The listing builds one solid part. Answer for the finished solid, in the listing's coordinates (mm). A direction names the side the tool comes from. Coordinates: 2 decimals unless noted, no trailing zeros. Order: outer loops, then holes, each group sorted by start corner. A loop starts at its lowest first (then second) coordinate and runs counter-clockwise, first axis right, second up.
```python
from build123d import *

# Parameters (mm, degrees)
BASE_FLANGE_SKETCH_R = 8
BASE_FLANGE_DEPTH    = 9
TOWER_DEPTH          = 30
SIDE_SLOT_DEPTH      = 21
CLIP_BOSS_DEPTH      = 6
CLIP_BOSS_DEPTH_BACK = 1
CLIP_SLOT_REACH      = 174.171
CLIP_SLOT_END_RADIUS = 15


with BuildPart() as part:
    # Base Flange Sketch → Base Flange (new body)
    with BuildSketch(Plane(origin=(0, 0, 0), x_dir=(1, 0, 0), z_dir=(0, 1, 0))):
        with BuildLine():
            Line((-27, 40), (27, 40))
            ThreePointArc((27, 40), (49.192388155, 49.192388155), (40, 27))
            Line((40, 27), (40, -27))
            ThreePointArc((40, -27), (49.192388155, -49.192388155), (27, -40))
            Line((27, -40), (-27, -40))
            ThreePointArc((-27, -40), (-49.192388155, -49.192388155), (-40, -27))
            Line((-40, -27), (-40, 27))
            ThreePointArc((-40, 27), (-49.192388155, 49.192388155), (-27, 40))
        make_face()
        with Locations(Location((-40, 40, 0), (0, 0, 270))):
            Circle(BASE_FLANGE_SKETCH_R, mode=Mode.SUBTRACT)
        with Locations(Location((40, 40, 0), (0, 0, 270))):
            Circle(BASE_FLANGE_SKETCH_R, mode=Mode.SUBTRACT)
        with Locations(Location((40, -40, 0), (0, 0, 270))):
            Circle(BASE_FLANGE_SKETCH_R, mode=Mode.SUBTRACT)
        with Locations(Location((-40, -40, 0), (0, 0, 270))):
            Circle(BASE_FLANGE_SKETCH_R, mode=Mode.SUBTRACT)
    extrude(amount=BASE_FLANGE_DEPTH)

    # Tower Profile Sketch → Tower (add, symmetric)
    with BuildSketch(Plane(origin=(0, 0, 0), x_dir=(0, 0, -1), z_dir=(1, 0, 0))):
        with BuildLine():
            Line((-30, 9), (-30, 125))
            ThreePointArc((-30, 125), (-21.213203436, 146.213203436), (0, 155))
            Line((0, 155), (0, 45))
            Line((0, 45), (30, 45))
            Line((30, 45), (30, 9))
            Line((30, 9), (-30, 9))
        make_face()
    extrude(amount=TOWER_DEPTH, both=True)

    # Lower Bore Profile Sketch → Lower Bore (revolve, cut)
    with BuildSketch(Plane(origin=(0, 0, 0), x_dir=(-1, 0, 0), z_dir=(0, 0, -1))):
        Polygon((30, 134), (10, 134), (10, 140), (-10, 140), (-10, 145), (-30, 145), (-30, 125), (30, 125), align=None)
    revolve(axis=Axis((30, 125, 0), (-1, 0, 0)), mode=Mode.SUBTRACT)

    # Upper Bore Profile Sketch → Upper Bore (revolve, cut)
    with BuildSketch(Plane(origin=(0, 0, 0), x_dir=(-1, 0, 0), z_dir=(0, 0, -1))):
        Polygon((30, 57), (15, 57), (15, 52), (-10, 52), (-10, 57), (-30, 57), (-30, 45), (30, 45), align=None)
    revolve(axis=Axis((-30, 45, 0), (1, 0, 0)), mode=Mode.SUBTRACT)

    # Side Slot Sketch → Side Slot (cut, symmetric)
    with BuildSketch(Plane(origin=(0, 0, 0), x_dir=(0, 0, -1), z_dir=(1, 0, 0))):
        with BuildLine():
            Line((19, 45), (30, 45))
            Line((30, 45), (30, 9))
            Line((30, 9), (0, 9))
            Line((0, 9), (0, 26))
            ThreePointArc((0, 26), (13.435028843, 31.564971157), (19, 45))
        make_face()
    extrude(amount=SIDE_SLOT_DEPTH, both=True, mode=Mode.SUBTRACT)

    # Clip Boss Sketch → Clip Boss (add, two sides: drawn at the far end of the back side and taken through both)
    with BuildSketch(Plane(origin=(0, 155, 0), x_dir=(1, 0, 0), z_dir=(0, 1, 0)).offset(-CLIP_BOSS_DEPTH_BACK)):
        with BuildLine():
            Line((-8, 0), (-4, 0))
            ThreePointArc((-4, 0), (0, -4), (4, 0))
            Line((4, 0), (8, 0))
            ThreePointArc((8, 0), (0, -8), (-8, 0))
        make_face()
    extrude(amount=CLIP_BOSS_DEPTH + CLIP_BOSS_DEPTH_BACK)

    # Clip Slot: up to this cylinder (the profile starts outside it)
    clip_slot_end = Plane(origin=(0, 125, 0), z_dir=(1, 0, 0)) * Cylinder(CLIP_SLOT_END_RADIUS, 379.342, mode=Mode.PRIVATE)
    # Clip Slot Sketch → Clip Slot (cut, up to the surface)
    with BuildSketch(Plane(origin=(0, 155, 0), x_dir=(1, 0, 0), z_dir=(0, 1, 0)), mode=Mode.PRIVATE) as clip_slot_sk1:
        with BuildLine():
            Line((-4, 0), (4, 0))
            ThreePointArc((4, 0), (0, -4), (-4, 0))
        make_face()
    clip_slot_tool1 = extrude(clip_slot_sk1.sketch, amount=-CLIP_SLOT_REACH, mode=Mode.PRIVATE) - clip_slot_end
    add(clip_slot_tool1.solids().sort_by_distance((0, 155, 1.697653))[0], mode=Mode.SUBTRACT)


solid = part.part
```
(1) Find section B-B (y = 11). Write down the section's boundary in (x, z).
(2) Find section D-D (z = 42). Write down the section's boundary in (x, y), and give its area (3 significant figures).
(3) Consider line 1 (Z direction, x = -39.5, y = 6.5); line 2 (X direction, y = 16, z = -3); line 3 (Y direction, x = -28, z = 6.5). Determine where each line is inside the solid, lowest interval first.
(4) Find section C-C (x = 35). Write down the section's boundary in (y, z) (3 decimals), and give its area (3 significant figures).
(5) For faces 4 (the face through (0, 4, -40)), 5 (the face through (0, 157, 8)), 6 (the face through (0, 66, 30)), 7 (the face through (-17, 145, 0)), determine the directions among +Z, -Z, +X, -X, +Y, -Y from which every point of the face is accessible in a straight line to the end or side of a thin tool.
(6) Each of these flat-tipped pins is pushed along its axis until it touches: pin 1 Ø16.5 at (y, z) = (125, 5) entering from +X; pin 2 Ø2 at (y, z) = (51, 7.5) entering from -X; pin 3 Ø9 at (y, z) = (20, -16) entering from -X; pin 4 Ø4 at (x, z) = (22, 15.5) entering from -Y. Where does it stop, or does it pass through?
(7) The mould has two halves that part along X. Classify faces 1 (the face through (30, 67, 6)), 2 (the face through (0, 161, 5)), 3 (the face through (1, 9, -1)): released by +X, released by -X, zero draft, split by the parting line, or undercut.
(8) Find section A-A (z = -25). Write down the section's boundary in (x, y).
Findings below:
1. outline: (-30, -30) - (-21, -30) - (-21, 0) - (21, 0) - (21, -30) - (30, -30) - (30, 30) - (-30, 30) - close
2. outline: (-52.85, 0) - (-47.75, 0) - (-47.75, 9) - (-52.85, 9) - close; (-32.25, 0) - (-27.15, 0) - (-27.15, 9) - (-32.25, 9) - close; (27.15, 0) - (32.25, 0) - (32.25, 9) - (27.15, 9) - close; (47.75, 0) - (52.85, 0) - (52.85, 9) - (47.75, 9) - close
2. area: 184 mm2
3. line 1: z = -52.99 to -47.98, -32.02 to 32.02, 47.98 to 52.99
3. line 2: x = -30 to -21, 21 to 30
3. line 3: y = 0 to 34.91, 55.09 to 118.78, 131.22 to 154.29
4. outline: (0, -52) - (9, -52) - (9, -46.245) - (0, -46.245) - close; (0, -33.755) - (9, -33.755) - (9, 33.755) - (0, 33.755) - close; (0, 46.245) - (9, 46.245) - (9, 52) - (0, 52) - close
4. area: 711 mm2
5. face 4: -Z, +Y, -Y
5. face 5: +Z, +Y
5. face 6: +Z, +X, -X, +Y
5. face 7: -Z, +X, -X, +Y
6. pin 1: stops at x = -10
6. pin 2: stops at x = -15
6. pin 3: stops at x = -30
6. pin 4: stops at y = 0
7. face 1: released by +X
7. face 2: zero draft
7. face 3: undercut
8. outline: (-40, 0) - (40, 0) - (40, 9) - (30, 9) - (30, 45) - (21, 45) - (21, 9) - (-21, 9) - (-21, 45) - (-30, 45) - (-30, 9) - (-40, 9) - close
